Input: dimensioned drawing with shaded views. Units: mm. Origin: part minimum x, y, z. Give positions to 0.01 mm unless a question says otherwise; leave off trailing zeros. Loops run counter-clockwise (first coordinate to the right, second up) from the corner with the lowest first, then second, coordinate; pieces in that order, holes last. Notation, with made-up numbers: M 64,11.25 L 70,11.25 A23 ccw 70,32.25 Z; hole C 40,79.25 d5. An arc over 180 degrees is marked long. Use CSV: the item, a comma, the result in double quotes. Start each with the question number.
Q1. Pin query (flat end, axial travel): pin 1 (1 mm diameter, centred on x = 3, z = 4, fed in from +Y); pin 2 (1.5 mm diameter, centred on x = 10, z = 0.5, fed in from -Y); pin 3 (1.5 mm diameter, centred on x = 6.5, z = 1, fed in from +Y). Return the tip coordinate at first contact, or that it passes through.
Q2. Pull-direction query (Y, two-part tool) for the marked faces 1, 2 and 3; classes: released by +Y, released by -Y, zero draft, split by the parting line, or undercut.
Q3. Material intervals for line 1 along Y through (x, z) = (11, 2.9); line 2 along X through (y, z) = (9, 0.85); line 3 along Y through (x, z) = (8.25, 1.7), sorted ascending.
Q4. Section A-A, the plane y = 11. Output: boundary loops of the cut face in (x, z), plus the area to 3 significant figures.
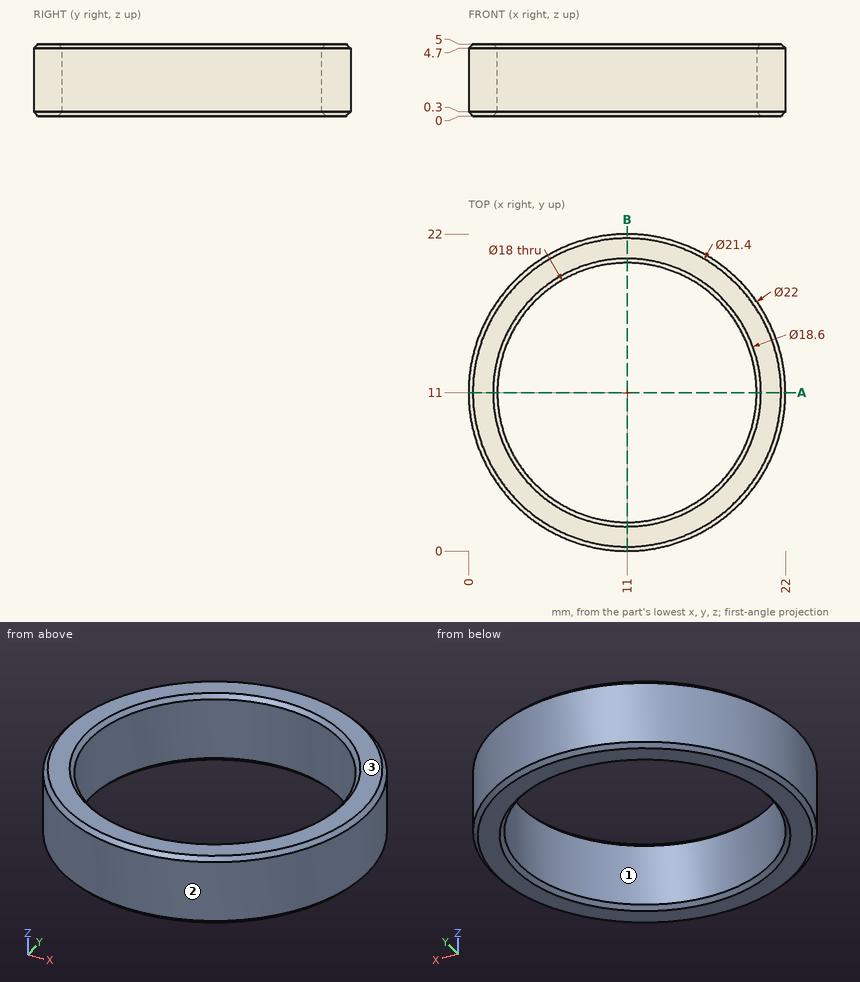
A:
1,pin 1,"y = 19.05"
1,pin 2,"y = 0"
1,pin 3,"y = 21.34"
2,face 1,"undercut"
2,face 2,"split by the parting line"
2,face 3,"zero draft"
3,line 1,"0 to 2, 20 to 22"
3,line 2,"0.18 to 2.23, 19.77 to 21.82"
3,line 3,"0.35 to 2.43, 19.57 to 21.65"
4,outline,"M 0,0.3 L 0.3,0 L 1.7,0 L 2,0.3 L 2,4.7 L 1.7,5 L 0.3,5 L 0,4.7 Z; M 20,0.3 L 20.3,0 L 21.7,0 L 22,0.3 L 22,4.7 L 21.7,5 L 20.3,5 L 20,4.7 Z"
4,area,"19.6 mm^2"
